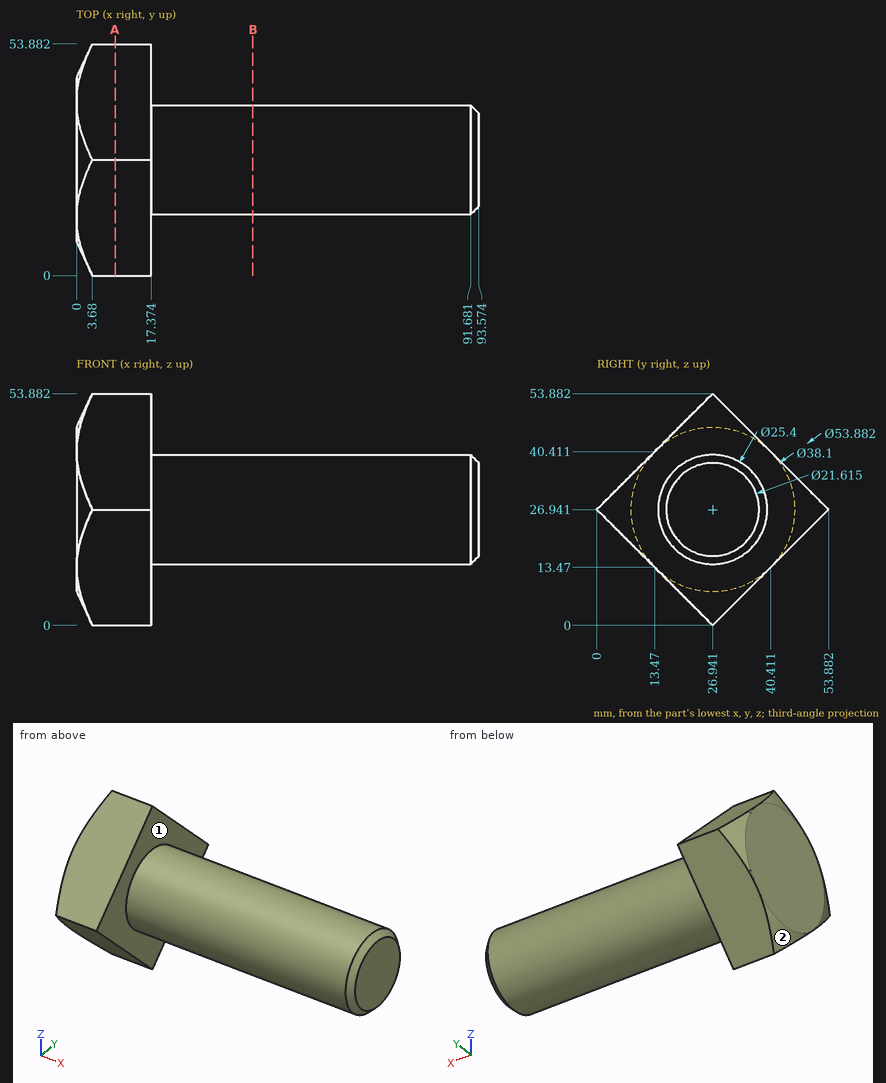
Job drawing, mm, ordinate dimensions from the low corner. One solid piece. A direction names the side the tool comes from. Coordinates: 2 decimals unless noted, no trailing zeros. Order: outer loops, then holes, each group sorted by start corner. A loop starts at its lowest first (then second) coordinate and runs counter-clockwise, first axis right, second up. Notation, with made-up numbers: M -39.75,-26.5 L -11.75,-26.5 A4 cw -11.75,-20.5 Z; hole C -4.5,84 d7. An arc over 180 degrees is marked long. Answer as CSV lines item,"result".
(1) Band-saw the part on B-B, the plane x = 41. List the corners of the cut face in (y, z).
Geometry says:
outline,"C 26.94,26.94 d25.4"
(2) Wall check: line 1 along X through (y, z) = (25, 40.5); line 2 along Z through (x, y) = (85, 27.5); line 3 along Y through (x, z) = (80, 33). Give the ranges that are in metal, low to high.
Geometry says:
line 1,"x = 0 to 17.37"
line 2,"z = 14.25 to 39.63"
line 3,"y = 15.78 to 38.1"
(3) 3-axis set-ups, long thin cutter, end or side, ignore diameter. For the marked faces 1 and 2: which of +Z, -Z, +X, -X, +Y, -Y reach the whole face in a straight line?
Geometry says:
face 1,"+X"
face 2,"-Z, -X"
(4) Band-saw the part on A-A, the plane x = 9. List the corners of the cut face in (y, z), then the cut area to 3 significant figures.
Geometry says:
outline,"M 0,26.94 L 26.94,0 L 53.88,26.94 L 26.94,53.88 Z"
area,"1,450 mm2"
(5) Flat gauge pins, fed straight in: pin 1 (2 mm diameter, centred on x = 35.5, z = 22.5, fed in from +Y) (1 decimal); pin 2 (10 mm diameter, centred on y = 7.5, z = 34.5, fed in from +X); pin 3 (4 mm diameter, centred on x = 10.5, z = 14.5, fed in from +Y). Where does each tip first touch, or does it go through?
Geometry says:
pin 1,"stops at y = 39.2"
pin 2,"stops at x = 17.37"
pin 3,"stops at y = 43.44"
